Here's the drawing with two shaded views (mm, measured from the low corner). I have some questions. A direction names the side the tool comes from. Round coordinates to 2 decimals unless told otherwise and drop trailing zeros. Loops run counter-clockwise (first coordinate to the right, second up) from the corner with the lowest first, then second, coordinate; pieces in that order, holes last. Notation, with made-up numbers: M 42.25,81.25 L 90.25,81.25 A31 ccw 90.25,112.25 Z; hole C -6.75,63.25 d6. An arc over 180 degrees is marked long. Answer as CSV lines item,"result".
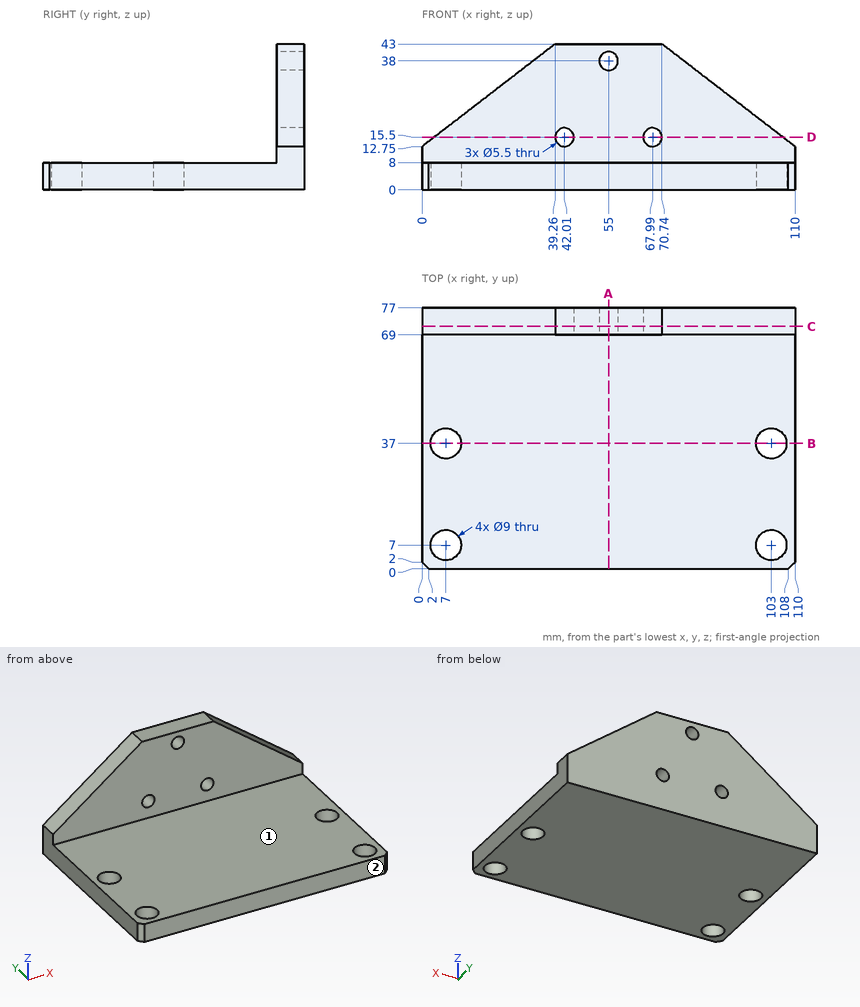
1. I want a section at A-A, the plane x = 55. Please give me the cut outline in (y, z).
Evaluation:
outline,"M 0,0 L 77,0 L 77,35.25 L 69,35.25 L 69,8 L 0,8 Z; M 69,40.75 L 77,40.75 L 77,43 L 69,43 Z"
2. I want a section at D-D, the plane z = 15.5. Please give me the cut outline in (x, y), and give its area (3 significant figures).
Evaluation:
outline,"M 3.57,69 L 39.26,69 L 39.26,77 L 3.57,77 Z; M 44.76,69 L 65.24,69 L 65.24,77 L 44.76,77 Z; M 70.74,69 L 106.43,69 L 106.43,77 L 70.74,77 Z"
area,"735 mm²"
3. I want a section at B-B, the plane y = 37. Please give me the cut outline in (x, z).
Evaluation:
outline,"M 0,0 L 2.5,0 L 2.5,8 L 0,8 Z; M 11.5,0 L 98.5,0 L 98.5,8 L 11.5,8 Z; M 107.5,0 L 110,0 L 110,8 L 107.5,8 Z"
4. For P1, Ø8, axis at x = 98.5, y = 58, coming from the +Z side; P2, Ø1, axis at x = 60.5, z = 21.5, coming from the -Y side; P3, Ø5.5, axis at x = 103, y = 37, coming from the -Z side (3 decimals), each with a flat end and sliding along its axis, tell me the tip position at first contact or that it passes through.
Evaluation:
P1,"stops at z = 8"
P2,"stops at y = 69"
P3,"passes through"
5. Which directions (+Z, -Z, +X, -X, +Y, -Y) give clear straight access to the entire face, cutting with the end or side of a thin tool? Please do the marked faces 1 and 2.
Evaluation:
face 1,"+Z, +X, -X, -Y"
face 2,"+Z, -Z, +X, -X, -Y"
6. If I drill on line 1 (Y direction, x = 103, z = 4.5); line 2 (X direction, y = 4.5, z = 7.5); line 3 (X direction, y = 72, z = 15) (1 decimal), over which ranges is the centre line in solid material (lowest first)? Write a range as [from, to].
Evaluation:
line 1,"y = [0, 2.5], [11.5, 32.5], [41.5, 77]"
line 2,"x = [0, 3.26], [10.74, 99.26], [106.74, 110]"
line 3,"x = [2.9, 39.3], [44.7, 65.3], [70.7, 107.1]"
7. I want a section at C-C, the plane y = 71.5. Please give me the cut outline in (x, z).
Evaluation:
outline,"M 0,0 L 110,0 L 110,12.75 L 70.74,43 L 39.26,43 L 0,12.75 Z; hole C 42.01,15.5 d5.5; hole C 55,38 d5.5; hole C 67.99,15.5 d5.5"
